For this review, take the finished solid that the model builds, in its own axes (mm). Face numbers are marked on the shaded views. A direction names the side the tool comes from. Coordinates: 2 decimals unless noted, no trailing zeros. Write each loop counter-clockwise with the first axis right and the second up, starting at its lowest first coordinate (ties: lowest second). Pieces come first, ordered by that corner, then holes.
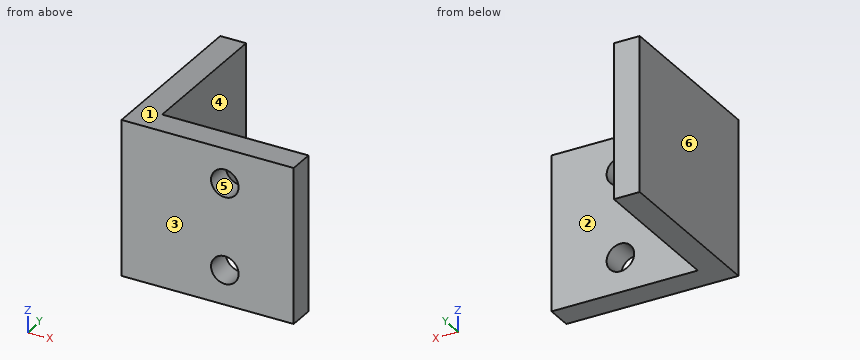
```python
from build123d import *

# Parameters (mm, degrees)
BOSS_EXTRUDE1_DEPTH = 90
SKETCH2_R           = 8
CUT_EXTRUDE1_DEPTH  = 90


with BuildPart() as part:
    # Sketch1 → Boss-Extrude1 (new body)
    with BuildSketch(Plane.XY):
        Polygon((0, 0), (0, 100), (15, 100), (15, 15), (100, 15), (100, 0), align=None)
    extrude(amount=BOSS_EXTRUDE1_DEPTH)

    # Sketch2 → Cut-Extrude1 (cut)
    with BuildSketch(Plane(origin=(0, 15, 0), x_dir=(1, 0, 0), z_dir=(0, 1, 0))):
        with Locations(Location((60, -20, 0), (0, 0, 270))):
            Circle(SKETCH2_R)
        with Locations(Location((60, -70, 0), (0, 0, 270))):
            Circle(SKETCH2_R)
    extrude(amount=-CUT_EXTRUDE1_DEPTH, mode=Mode.SUBTRACT)


solid = part.part
```
Q1. Tool access review of the marked faces 1 and 2: name each direction out of +Z, -Z, +X, -X, +Y, -Y from which nothing blocks a thin tool from reaching the whole face with its end or side.
Ans:
face 1: +Z, +X, -X, +Y, -Y
face 2: +Z, -Z, +X, +Y
Q2. Add section C-C (z = 60). State the section outline as (x, y) points, then the cut area to 4 significant figures.
Ans:
outline: (0, 0) - (100, 0) - (100, 15) - (15, 15) - (15, 100) - (0, 100) - close
area: 2,775 mm2
Q3. Add section D-D (y = 81.5). State the section outline as (x, z) points, then the cut area to 3 significant figures.
Ans:
outline: (0, 0) - (15, 0) - (15, 90) - (0, 90) - close
area: 1,350 mm2
Q4. Add section B-B (y = 8.5). State the section outline as (x, z) points, then the cut area to 3 significant figures.
Ans:
outline: (0, 0) - (100, 0) - (100, 90) - (0, 90) - close; hole circle Ø16 at (60, 20); hole circle Ø16 at (60, 70)
area: 8,600 mm2
Q5. For probe 1 along X at (y, z) = (11.5, 20); probe 2 along X at (y, z) = (94, 59.5), list the stretches that pass through material, from the lowest coordinate up.
Ans:
probe 1: x = 0 to 52, 68 to 100
probe 2: x = 0 to 15
Q6. Add section A-A (z = 70). State the section outline as (x, y) points, then the cut area to 4 significant figures.
Ans:
outline: (0, 0) - (52, 0) - (52, 15) - (15, 15) - (15, 100) - (0, 100) - close; (68, 0) - (100, 0) - (100, 15) - (68, 15) - close
area: 2,535 mm2
Q7. Draft analysis for pull direction X (two halves, no side actions). For the marked faces 3, 4, 5 and 6, state which applies: +X half, -X half, draft (parallel to the pull), parting line (faces both ways), or undercut.
Ans:
face 3: draft
face 4: +X half
face 5: undercut
face 6: -X half
Q8. Clearance check with flat-ended pins moving along their axes: pin 1 Ø2 at (x, z) = (37, 37.5) entering from +Y; pin 2 Ø4 at (y, z) = (87, 43.5) entering from +X. State where each tip first meets the part, or that it passes through.
Ans:
pin 1: stops at y = 15
pin 2: stops at x = 15
